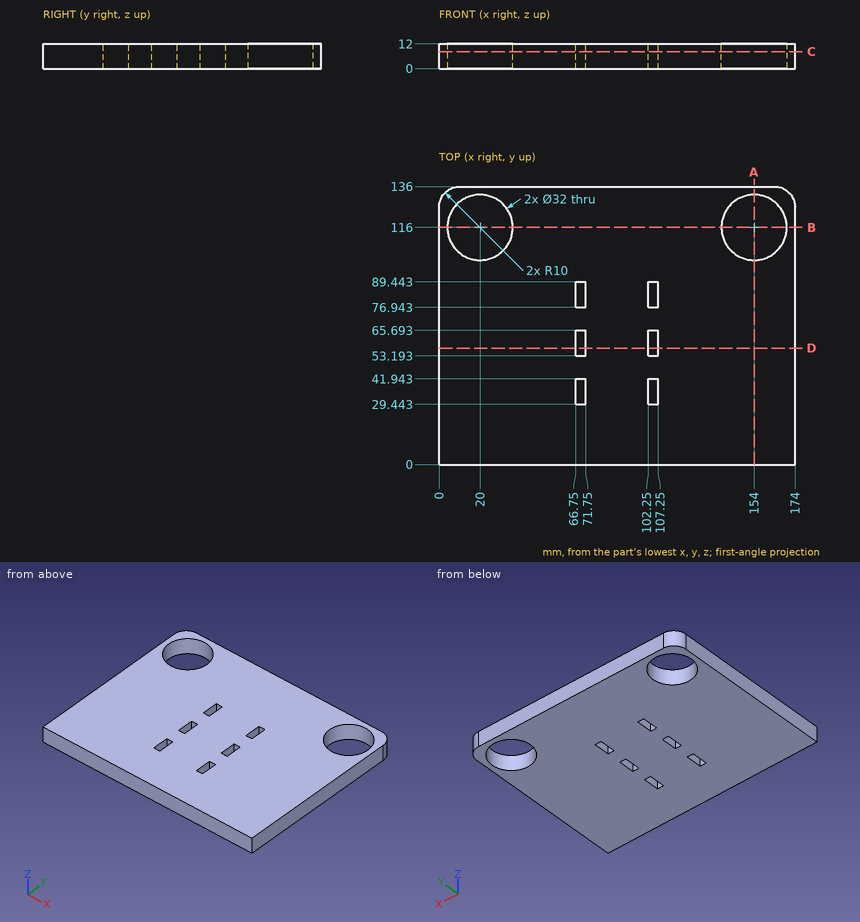
The figure shows three views and two pictorial views of one solid part (mm, origin at its lowest corner). Answer the questions. Give positions to 0.01 mm unless a question says otherwise; leave off trailing zeros. Order: outer loops, then holes, each group sorted by start corner. A loop starts at its lowest first (then second) coordinate and runs counter-clockwise, first axis right, second up. Notation, with made-up numbers: (-34.75, 17) -> (15.25, 17) arc R26 ccw to (15.25, 52) -> close; hole circle Ø4 at (79.5, 37). An arc over 180 degrees is marked (long way). Answer as CSV lines item,"result". Start each with the question number.
(1) Consider line 1 along X through (y, z) = (89, 5); line 2 along Y through (x, z) = (20, 5.75); line 3 along X through (y, z) = (111, 10). Determine where each line is inside the solid, lowest interval first.
(2) Section B-B, the plane y = 116 is taken. Write down the section's boundary in (x, z).
(3) Section C-C, the plane z = 8.25 is taken. Give the number of separate pieces and of enclosed holes in the cut face, plus the area to 3 significant figures.
(4) Section A-A, the plane x = 154 is taken. Write down the section's boundary in (y, z), plus the area to 3 significant figures.
(5) Section D-D, the plane y = 57 is taken. Write down the section's boundary in (x, z).
Entries:
1,line 1,"0 to 66.75, 71.75 to 102.25, 107.25 to 174"
1,line 2,"0 to 100, 132 to 136"
1,line 3,"0 to 4.8, 35.2 to 138.8, 169.2 to 174"
2,outline,"(0, 0) -> (4, 0) -> (4, 12) -> (0, 12) -> close; (36, 0) -> (138, 0) -> (138, 12) -> (36, 12) -> close; (170, 0) -> (174, 0) -> (174, 12) -> (170, 12) -> close"
3,separate pieces,"1"
3,enclosed holes,"8"
3,area,"21,600 mm²"
4,outline,"(0, 0) -> (100, 0) -> (100, 12) -> (0, 12) -> close; (132, 0) -> (136, 0) -> (136, 12) -> (132, 12) -> close"
4,area,"1,250 mm²"
5,outline,"(0, 0) -> (66.75, 0) -> (66.75, 12) -> (0, 12) -> close; (71.75, 0) -> (102.25, 0) -> (102.25, 12) -> (71.75, 12) -> close; (107.25, 0) -> (174, 0) -> (174, 12) -> (107.25, 12) -> close"
